```python
from build123d import *

# Parameters (mm, degrees)
SKETCH1_W           = 60
SKETCH1_H           = 60
BOSS_EXTRUDE1_DEPTH = 180
M12_TAPPED_HOLE1_D  = 10.2


with BuildPart() as part:
    # Sketch1 → Boss-Extrude1 (new body)
    with BuildSketch(Plane.XY):
        Rectangle(SKETCH1_W, SKETCH1_H)
    extrude(amount=BOSS_EXTRUDE1_DEPTH)

    # M12 Tapped Hole1 (through all)
    with Locations(Plane(origin=(0, 30, 0), x_dir=(1, 0, 0), z_dir=(0, 1, 0))):
        with Locations((0, -22.5), (0, -157.5)):
            Hole(M12_TAPPED_HOLE1_D / 2)


solid = part.part
```
The listing builds one solid part. Answer for the finished solid, in the listing's coordinates (mm). Give positions to 0.01 mm unless a question says otherwise; leave off trailing zeros. Loops run counter-clockwise (first coordinate to the right, second up) from the corner with the lowest first, then second, coordinate; pieces in that order, holes last. Notation, with made-up numbers: (-2, -11.75) - (28, -11.75) arc R26 ccw to (28, 27.25) - close; hole circle Ø8 at (-22, -38). An arc over 180 degrees is marked (long way). Answer as CSV lines item,"result". Start each with the question number.
Item 1: Find the intervals of material crossed by line 1 (Z direction, x = 0, y = -10); line 2 (X direction, y = -1.5, z = 157.5); line 3 (Z direction, x = 3, y = 17), in increasing order. Write a range as from..to.
Item 2: The mould has two halves that part along Z. Classify faces 1 (the face through (1.106, -0.42, 162.479)), 2 (the face through (1.106, -0.42, 27.479)), 3 (the face through (30, 0, 89)), 4 (the face through (0, 0, 0)): +Z half, -Z half, draft (parallel to the pull), parting line (faces both ways), or undercut.
Item 3: A cutting plane is placed at B-B on y = 11. Determine the outline of the cut face in (x, z).
Item 4: A cutting plane is placed at A-A on x = 0. Determine the outline of the cut face in (y, z).
Item 5: This flat-tipped pin is pushed along its axis until it touches: pin 1 (2 mm diameter, centred on x = 4, y = -23.5, fed in from -Z). Where does it stop, or does it pass through?
Found:
1,line 1,"z = 0..17.4, 27.6..152.4, 162.6..180"
1,line 2,"x = -30..-5.1, 5.1..30"
1,line 3,"z = 0..18.38, 26.62..153.38, 161.62..180"
2,face 1,"undercut"
2,face 2,"undercut"
2,face 3,"draft"
2,face 4,"-Z half"
3,outline,"(-30, 0) - (30, 0) - (30, 180) - (-30, 180) - close; hole circle Ø10.2 at (0, 22.5); hole circle Ø10.2 at (0, 157.5)"
4,outline,"(-30, 0) - (30, 0) - (30, 17.4) - (-30, 17.4) - close; (-30, 27.6) - (30, 27.6) - (30, 152.4) - (-30, 152.4) - close; (-30, 162.6) - (30, 162.6) - (30, 180) - (-30, 180) - close"
5,pin 1,"stops at z = 0"
